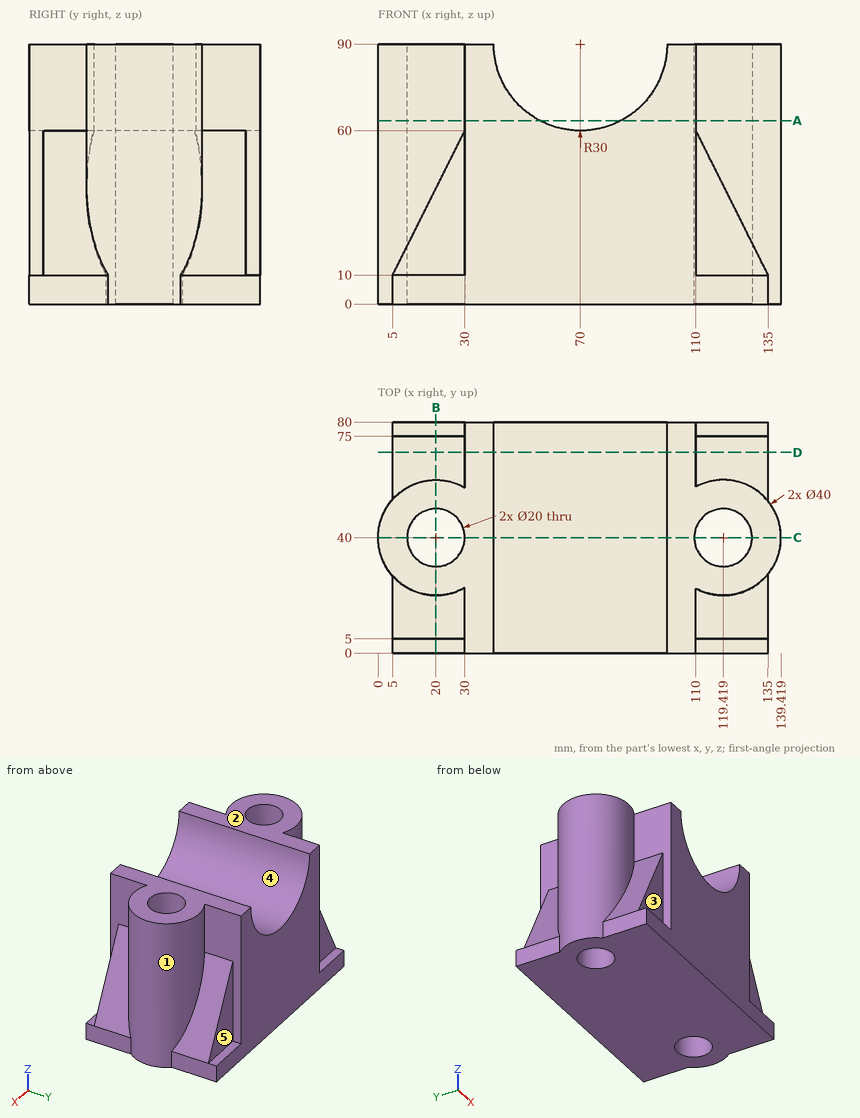
For this review, use the dimensioned drawing (mm, ordinates from the lowest corner) and the shaded views. A direction names the side the tool comes from. Give positions to 0.01 mm unless a question says otherwise; leave off trailing zeros. Write each loop counter-clockwise with the first axis right and the second up, starting at its lowest first coordinate (ties: lowest second). Pieces come first, ordered by that corner, then holes.
(1) To check wall thickness, follow L1, parallel to X at y = 33, z = 47 (1 decimal); L2, parallel to X at y = 42, z = 41; L3, parallel to Y at x = 20, z = 39. State the ranges of each line that lie inside material, in increasing order.
(2) Consider section D-D, the plane y = 69.5. Give the boundary of the cut face in (x, z).
(3) Consider section A-A, the plane z = 63.5. Give the boundary of the cut face in (x, y), and give its area (3 significant figures).
(4) Consider section C-C, the plane y = 40. Give the boundary of the cut face in (x, z).
(5) Consider section B-B, the plane x = 20. Give the boundary of the cut face in (y, z), and give its area (3 significant figures).
(6) Tool access review of the marked faces 3, 4 and 5: name each direction out of +Z, -Z, +X, -X, +Y, -Y from which nothing blocks a thin tool from reaching the whole face with its end or side.
(7) The part is to be moulded in two halves that separate along X. For the marked faces 1 and 2, say which applies: released by +X, released by -X, zero draft, split by the parting line, or undercut.
(8) For P1, Ø3, axis at y = 19.5, z = 25.5, coming from the +X side; P2, Ø12.5, axis at x = 122.5, z = 38.5, coming from the +Y side; P3, Ø5, axis at x = 105.5, z = 35.5, coming from the -Y side; P4, Ø2, axis at x = 123.5, z = 22, coming from the -Y side, all flat-tipped, find the tip position at first contact; note any pin that passes through.
Returned:
1. L1: x = 1.3 to 12.9, 27.1 to 112.3, 126.6 to 138.2
1. L2: x = 0.1 to 10.2, 29.8 to 109.62, 129.22 to 139.32
1. L3: y = 5 to 30, 50 to 75
2. outline: (5, 0) - (135, 0) - (135, 10) - (110, 60) - (110, 90) - (100, 90) arc R30 cw to (40, 90) - (30, 90) - (30, 60) - (5, 10) - close
3. outline: (30, 0) - (55.94, 0) - (55.94, 80) - (30, 80) - (30, 57.32) arc R20 ccw (long way) to (30, 22.68) - close; (84.06, 0) - (110, 0) - (110, 22.36) arc R20 ccw (long way) to (110, 57.64) - (110, 80) - (84.06, 80) - close; hole circle Ø20 at (20, 40); hole circle Ø20 at (119.42, 40)
3. area: 5,520 mm2
4. outline: (0, 0) - (10, 0) - (10, 90) - (0, 90) - close; (30, 0) - (109.42, 0) - (109.42, 90) - (100, 90) arc R30 cw to (40, 90) - (30, 90) - close; (129.42, 0) - (139.42, 0) - (139.42, 90) - (129.42, 90) - close
5. outline: (0, 0) - (30, 0) - (30, 90) - (20, 90) - (20, 40) - (5, 40) - (5, 10) - (0, 10) - close; (50, 0) - (80, 0) - (80, 10) - (75, 10) - (75, 40) - (60, 40) - (60, 90) - (50, 90) - close
5. area: 3,100 mm2
6. face 3: +Z, -X, -Y
6. face 4: +Z, +Y, -Y
6. face 5: +Z, +X, +Y
7. face 1: undercut
7. face 2: zero draft
8. P1: stops at x = 128
8. P2: stops at y = 75
8. P3: stops at y = 0
8. P4: stops at y = 5
